For this review, take the finished solid that the model builds, in its own axes (mm). A direction names the side the tool comes from. Round coordinates to 2 decimals unless told otherwise and drop trailing zeros. Order: outer loops, then holes, each group sorted by start corner. A loop starts at its lowest first (then second) coordinate and runs counter-clockwise, first axis right, second up.
```python
from build123d import *

# Parameters (mm, degrees)
EXTRUDE_1_DEPTH          = 5
SKETCH_4_R               = 27.5
CUT_EXTRUDE_4_DEPTH      = 20
SKETCH_5_W               = 104
SKETCH_5_H               = 9
EXTRUDE_2_DEPTH          = 150
CUT_EXTRUDE_5_DEPTH      = 171.582117426
CUT_EXTRUDE_5_DEPTH_BACK = 171.582117426
SKETCH_6_R               = 5


with BuildPart() as part:
    # 草图1 → 凸台-拉伸1 (new body)
    with BuildSketch(Plane.XY):
        Polygon((-50.354639151, -47.265777393), (-50.354639151, -53.645360849), (-50.354639151, -60.995360849), (53.645360849, -60.995360849), (53.645360849, -53.645360849), (53.645360849, 50.354639151), (-50.354639151, 50.354639151), align=None)
    extrude(amount=EXTRUDE_1_DEPTH)

    # 草图4 → 切除-拉伸4 (cut)
    with BuildSketch(Plane.XY.offset(5)):
        Circle(SKETCH_4_R)
    extrude(amount=-CUT_EXTRUDE_4_DEPTH, mode=Mode.SUBTRACT)

    # 草图5 → 凸台-拉伸2 (add)
    with BuildSketch(Plane(origin=(0, 0, 0), x_dir=(-1, 0, 0), z_dir=(0, 0, -1))):
        with Locations((-1.645360849, -56.495360849)):
            Rectangle(SKETCH_5_W, SKETCH_5_H)
    extrude(amount=EXTRUDE_2_DEPTH)

    # 草图6 → 切除-拉伸5 (cut, two sides: drawn at the far end of the back side and taken through both)
    with BuildSketch(Plane(origin=(0, 0, 0), x_dir=(-1, 0, 0), z_dir=(0, 0, -1)).offset(-CUT_EXTRUDE_5_DEPTH_BACK)):
        with Locations((-42.426406871, 42.426406871)):
            Circle(SKETCH_6_R)
        with Locations((42.426406871, 42.426406871)):
            Circle(SKETCH_6_R)
        with Locations((42.426406871, -42.426406871)):
            Circle(SKETCH_6_R)
        with Locations((-42.426406871, -42.426406871)):
            Circle(SKETCH_6_R)
    extrude(amount=CUT_EXTRUDE_5_DEPTH + CUT_EXTRUDE_5_DEPTH_BACK, mode=Mode.SUBTRACT)


solid = part.part
```
Q1. Mouldability with a two-part tool opening along X and no side actions: class faces 3 (the face through (-50.355, -55, -49)), 4 (the face through (53.645, -55, -49)), 5 (the face through (2, -60.995, -71)), 6 (the face through (-45.114, 46.642, 2.535)) as +X half, -X half, draft (parallel to the pull), parting line (faces both ways), or undercut.
Q2. Take a section at C-C, the plane z = -135.5. State the section outline as (x, y) points.
Q3. Take a section at A-A, the plane y = 0. State the section outline as (x, z) points, plus the area to 3 significant figures.
Q4. Take a section at B-B, the plane x = 0. State the section outline as (y, z) points.
Q5. Take a section at D-D, the plane x = 29.5. State the section outline as (y, z) points, plus the area to 3 significant figures.
Q6. Tool access review of faces 1 (the face through (-45.1, -38.2, 2.5)), 2 (the face through (2, -51.995, -74)): name each direction out of +Z, -Z, +X, -X, +Y, -Y from which nothing blocks a thin tool from reaching the whole face with its end or side.
Q7. Clearance check with flat-ended pins moving along their axes: pin 1 (16 mm diameter, centred on x = -42.43, y = 42.43, fed in from +Z); pin 2 (1.5 mm diameter, centred on x = -25.5, y = -32, fed in from -Z). State where each tip first meets the part, or that it passes through.
Q8. Wall thickness on line 1 (Y direction, x = 7, z = -87.5); line 2 (Z direction, x = 32, y = -30.5); line 3 (Y direction, x = 0, z = 1.6): over which ranges is each line inside the solid? List them lowest first.
Working result:
1. face 3: -X half
1. face 4: +X half
1. face 5: draft
1. face 6: undercut
2. outline: (-50.35, -61) - (53.65, -61) - (53.65, -52) - (-50.35, -52) - close
3. outline: (-50.35, 0) - (-27.5, 0) - (-27.5, 5) - (-50.35, 5) - close; (27.5, 0) - (53.65, 0) - (53.65, 5) - (27.5, 5) - close
3. area: 245 mm2
4. outline: (-61, -150) - (-52, -150) - (-52, 0) - (-27.5, 0) - (-27.5, 5) - (-61, 5) - close; (27.5, 0) - (50.35, 0) - (50.35, 5) - (27.5, 5) - close
5. outline: (-61, -150) - (-52, -150) - (-52, 0) - (50.35, 0) - (50.35, 5) - (-61, 5) - close
5. area: 1,910 mm2
6. face 1: +Z, -Z
6. face 2: -Z, +X, -X, +Y
7. pin 1: stops at z = 5
7. pin 2: stops at z = 0
8. line 1: y = -61 to -52
8. line 2: z = 0 to 5
8. line 3: y = -61 to -27.5, 27.5 to 50.35
